Here's how the part is built. I have some questions about the finished solid (model axes, mm). A direction names the side the tool comes from. Give positions to 0.01 mm unless a question says otherwise; leave off trailing zeros. Loops run counter-clockwise (first coordinate to the right, second up) from the corner with the lowest first, then second, coordinate; pieces in that order, holes last.
Q1. I need wall thicknesses on line 1 (Y direction, x = -6.5, z = 0.8); line 2 (Y direction, x = 25, z = 0.2); line 3 (Y direction, x = 34.5, z = 0.2). Which ranges of each line are inside material? Lowest first, please.
Q2. If we section it at D-D (y = 95): Please give me the cut outline in (x, z), plus the area to 3 significant figures.
Q3. For faces 1 (the face through (38.36, 77.6, 0.01)), 2 (the face through (-62.96, 47.39, 0.01)), which set-ups out of +Z, -Z, +X, -X, +Y, -Y let a thin tool reach every point of the face, with its end or its side?
Q4. If we section it at C-C (z = 0.65): Please give me the cut outline in (x, y), plus the area to 3 significant figures.
Q5. We'd pull the mould along Y, two halves only. Please class faces 3 (the face through (-58.7, 104.6, 0)), 4 (the face through (-62.965, 127.462, 0.014)), 5 (the face through (-10, 87, -1)): +Y half, -Y half, draft (parallel to the pull), parting line (faces both ways), or undercut.
Q6. Will this pin go through, and if not, where does the flat tip stop? P1, Ø5, axis at x = -55.5, y = 119.93, coming from the -Z side.
Q7. If we section it at B-B (x = -55.5): Please give me the cut outline in (y, z), plus the area to 3 significant figures.
Q8. If we section it at A-A (x = 24): Please give me the cut outline in (y, z), plus the area to 3 significant figures.
from build123d import *

# Parameters (mm, degrees)
EXTRUDE_1_DEPTH              = 1
HOLE_WIZARD_M6_1_D           = 6.6
HOLE_WIZARD_M6_1_CBORE_D     = 11
HOLE_WIZARD_M6_1_CBORE_DEPTH = 6.4
SKETCH_27_W                  = 153
SKETCH_27_H                  = 120
EXTRUDE_3_DEPTH              = 2
HOLE_WIZARD_M5_2_D           = 4.2
HOLE_WIZARD_M5_2_DEPTH       = 14
HOLE_WIZARD_M5_2_TIP         = 1.2618073
SKETCH_15_W                  = 112.889805259
SKETCH_15_H                  = 130.002769253
CUT_EXTRUDE_1_DEPTH          = 512.721848273
SKETCH_16_R                  = 10
CUT_EXTRUDE_2_DEPTH          = 2
SKETCH_18_R                  = 10
CUT_EXTRUDE_4_DEPTH          = 2
SKETCH_28_W                  = 266.209573984
SKETCH_28_H                  = 254.96875003
CUT_EXTRUDE_7_DEPTH          = 512.721848273
SKETCH_29_W                  = 20
SKETCH_29_H                  = 197
EXTRUDE_4_DEPTH              = 2
SKETCH_30_W                  = 160
SKETCH_30_H                  = 28
EXTRUDE_5_DEPTH              = 2
SKETCH_31_W                  = 160
SKETCH_31_H                  = 323
CUT_EXTRUDE_8_DEPTH          = 471.473431768
SKETCH_32_W                  = 27
SKETCH_32_H                  = 140
CUT_EXTRUDE_9_DEPTH          = 164.022237747
SKETCH_33_R                  = 10
EXTRUDE_6_DEPTH              = 2
EXTRUDE_7_DEPTH              = 2
HOLE_WIZARD_M6_2_D           = 6.6
HOLE_WIZARD_M6_2_CBORE_D     = 11
HOLE_WIZARD_M6_2_CBORE_DEPTH = 6.4
SKETCH_38_W                  = 13
SKETCH_38_H                  = 160
CUT_EXTRUDE_10_DEPTH         = 10
SKETCH_39_W                  = 50
SKETCH_39_H                  = 110.0725
EXTRUDE_8_DEPTH              = 2
SKETCH_40_W                  = 120
SKETCH_40_H                  = 49.9275
CUT_EXTRUDE_11_DEPTH         = 185.727502013
HOLE_WIZARD_5_5_5_5_1_D      = 5.5
MOVE_FACE_1_BY               = 7.5
MOVE_FACE_2_BY               = 7.5
FILLET_4_R                   = 10
SKETCH_44_OUTSIDE_W          = 214.212
SKETCH_44_OUTSIDE_H          = 169.284
SKETCH_44_OUTSIDE_W_2        = 110
SKETCH_44_OUTSIDE_H_2        = 85
CUT_EXTRUDE_12_DEPTH         = 191.47440773
CHAMFER_1_SIZE               = 5
HOLE_WIZARD_5_5_5_5_2_D      = 5.5
CUT_EXTRUDE_13_DEPTH         = 10


with BuildPart() as part:
    # Model → 凸台-拉伸1 (new, symmetric)
    with BuildSketch(Plane.XY):
        with BuildLine():
            Line((186.507023758, 241.511944981), (58.910891188, 92.809685219))
            ThreePointArc((58.910891188, 92.809685219), (57.122071441, 89.769692994), (56.5, 86.297740238))
            Line((56.5, 86.297740238), (56.5, 0))
            Line((56.5, 0), (-73.5, 0))
            ThreePointArc((-73.5, 0), (-80.571067812, 2.928932188), (-83.5, 10))
            Line((-83.5, 10), (-83.5, 335))
            Line((-83.5, 335), (59.5, 335))
            ThreePointArc((59.5, 335), (66.571067812, 337.928932188), (69.5, 345))
            Line((69.5, 345), (69.5, 435))
            Line((69.5, 435), (259.5, 435))
            ThreePointArc((259.5, 435), (266.571067812, 432.071067812), (269.5, 425))
            Line((269.5, 425), (269.5, 255))
            ThreePointArc((269.5, 255), (266.571067812, 247.928932188), (259.5, 245))
            Line((259.5, 245), (194.09613257, 245))
            ThreePointArc((194.09613257, 245), (189.91997703, 244.086238215), (186.507023758, 241.511944981))
        make_face()
    extrude(amount=EXTRUDE_1_DEPTH, both=True)

    # M6 六角凹头螺钉的柱形沉头孔1 (through all)
    with Locations(Plane(origin=(0, 0, -1), x_dir=(-1, 0, 0), z_dir=(0, 0, -1))):
        with Locations((16.5, 157), (-9.5, 235), (-9.5, 157), (16.5, 235)):
            CounterBoreHole(HOLE_WIZARD_M6_1_D / 2, HOLE_WIZARD_M6_1_CBORE_D / 2, HOLE_WIZARD_M6_1_CBORE_DEPTH)

    # 草图27 → 凸台-拉伸3 (add)
    with BuildSketch(Plane.XY.offset(1)):
        with Locations((-7, 375)):
            Rectangle(SKETCH_27_W, SKETCH_27_H)
    extrude(amount=-EXTRUDE_3_DEPTH)

    # M5 螺纹孔2
    with Locations(Plane.XY.offset(1)):
        with Locations((-60.5, 390), (27.5, 405), (47.5, 265), (-32.5, 270)):
            Hole(HOLE_WIZARD_M5_2_D / 2, depth=HOLE_WIZARD_M5_2_DEPTH)
            with Locations((0, 0, -(HOLE_WIZARD_M5_2_DEPTH + HOLE_WIZARD_M5_2_TIP / 2))):  # 118° drill point
                Cone(0, HOLE_WIZARD_M5_2_D / 2, HOLE_WIZARD_M5_2_TIP, mode=Mode.SUBTRACT)

    # 草图15 → 切除-拉伸1 (cut, through all)
    with BuildSketch(Plane.XY.offset(1)):
        with Locations((112.94490263, 131.998615374)):
            Rectangle(SKETCH_15_W, SKETCH_15_H)
    extrude(amount=-CUT_EXTRUDE_1_DEPTH, mode=Mode.SUBTRACT)

    # 草图16 → 切除-拉伸2 (cut)
    with BuildSketch(Plane.XY.offset(1)):
        with Locations((-13.5, 25)):
            Circle(SKETCH_16_R)
    cut_extrude_2 = extrude(amount=-CUT_EXTRUDE_2_DEPTH, mode=Mode.SUBTRACT)

    # 草图18 → 切除-拉伸4 (cut)
    with BuildSketch(Plane.XY.offset(1)):
        with Locations((244.5, 340)):
            Circle(SKETCH_18_R)
    extrude(amount=-CUT_EXTRUDE_4_DEPTH, mode=Mode.SUBTRACT)

    # 草图28 → 切除-拉伸7 (cut, through all)
    with BuildSketch(Plane.XY.offset(1)):
        with Locations((209.604786992, 307.515624985)):
            Rectangle(SKETCH_28_W, SKETCH_28_H)
    extrude(amount=-CUT_EXTRUDE_7_DEPTH, mode=Mode.SUBTRACT)

    # 草图29 → 凸台-拉伸4 (add)
    with BuildSketch(Plane.XY.offset(1)):
        with Locations((66.5, 98.5)):
            Rectangle(SKETCH_29_W, SKETCH_29_H)
    extrude(amount=-EXTRUDE_4_DEPTH)

    # 草图30 → 凸台-拉伸5 (add)
    with BuildSketch(Plane.XY.offset(1)):
        with Locations((-3.5, 449)):
            Rectangle(SKETCH_30_W, SKETCH_30_H)
    extrude(amount=-EXTRUDE_5_DEPTH)

    # 镜向1: 切除-拉伸2 across plane
    add(cut_extrude_2.mirror(Plane.ZX.offset(231.5)), mode=Mode.SUBTRACT)

    # 草图31 → 切除-拉伸8 (cut, through all)
    with BuildSketch(Plane.XY.offset(1)):
        with Locations((-3.5, 301.5)):
            Rectangle(SKETCH_31_W, SKETCH_31_H)
    extrude(amount=-CUT_EXTRUDE_8_DEPTH, mode=Mode.SUBTRACT)

    # 草图32 → 切除-拉伸9 (cut, through all)
    with BuildSketch(Plane.XY.offset(1)):
        with Locations((63, 70)):
            Rectangle(SKETCH_32_W, SKETCH_32_H)
    extrude(amount=-CUT_EXTRUDE_9_DEPTH, mode=Mode.SUBTRACT)

    # 草图33 → 凸台-拉伸6 (add)
    with BuildSketch(Plane.XY.offset(1)):
        with Locations((-13.5, 25)):
            Circle(SKETCH_33_R)
    extrude(amount=-EXTRUDE_6_DEPTH)

    # 草图37 → 凸台-拉伸7 (add)
    with BuildSketch(Plane.XY.offset(1)):
        with BuildLine():
            Line((49.5, 0), (-73.5, 0))
            ThreePointArc((-73.5, 0), (-80.571067812, 2.928932188), (-83.5, 10))
            Line((-83.5, 10), (-83.5, -20))
            Line((-83.5, -20), (49.5, -20))
            Line((49.5, -20), (49.5, 0))
        make_face()
    extrude(amount=-EXTRUDE_7_DEPTH)

    # M6 六角凹头螺钉的柱形沉头孔2 (through all)
    with Locations(Plane.XY.offset(1)):
        with Locations((-40.5, -10), (-40.5, 15), (19.5, 15), (19.5, -10)):
            CounterBoreHole(HOLE_WIZARD_M6_2_D / 2, HOLE_WIZARD_M6_2_CBORE_D / 2, HOLE_WIZARD_M6_2_CBORE_DEPTH)

    # 草图38 → 切除-拉伸10 (cut)
    with BuildSketch(Plane.XY.offset(1)):
        with Locations((-77, 60)):
            Rectangle(SKETCH_38_W, SKETCH_38_H)
    extrude(amount=-CUT_EXTRUDE_10_DEPTH, mode=Mode.SUBTRACT)

    # 草图39 → 凸台-拉伸8 (add)
    with BuildSketch(Plane.XY.offset(1)):
        with Locations((-95.5, 84.96375)):
            Rectangle(SKETCH_39_W, SKETCH_39_H)
    extrude(amount=-EXTRUDE_8_DEPTH)

    # 草图40 → 切除-拉伸11 (cut, through all)
    with BuildSketch(Plane(origin=(0, 0, -1), x_dir=(-1, 0, 0), z_dir=(0, 0, -1))):
        with Locations((10.5, 4.96375)):
            Rectangle(SKETCH_40_W, SKETCH_40_H)
    extrude(amount=-CUT_EXTRUDE_11_DEPTH, mode=Mode.SUBTRACT)

    # Ø5.5 (5.5) 直径孔1 (through all)
    with Locations(Plane.XY.offset(1)):
        with Locations((-87.5, 57.4275), (-112.5, 57.4275), (-112.5, 117.4275), (-87.5, 117.4275)):
            Hole(HOLE_WIZARD_5_5_5_5_1_D / 2)

    # Move Face 1: a face moved outward by 7.5
    extrude(part.faces().sort_by_distance((-35.5, 29.9275, 0))[0], amount=MOVE_FACE_1_BY, dir=(0, -1, 0))

    # Move Face 2: a face moved outward by 7.5
    extrude(part.faces().sort_by_distance((-35.5, 140, 0))[0], amount=MOVE_FACE_2_BY, dir=(0, 1, 0))

    # 圆角4
    fillet_4_edges = [part.edges().sort_by_distance(p)[0] for p in [
        (49.5, 147.5, 0),
        (-120.5, 147.5, 0),
        (-120.5, 22.4275, 0),
        (49.5, 22.4275, 0),
    ]]
    fillet(fillet_4_edges, radius=FILLET_4_R)

    # 草图44 outside → 切除-拉伸12 (cut, through all)
    with BuildSketch(Plane.XY.offset(1)):
        with Locations((-35.5, 84.964)):
            Rectangle(SKETCH_44_OUTSIDE_W, SKETCH_44_OUTSIDE_H)
        with Locations((-10.5, 87.4275)):
            Rectangle(SKETCH_44_OUTSIDE_W_2, SKETCH_44_OUTSIDE_H_2, mode=Mode.SUBTRACT)
    extrude(amount=-CUT_EXTRUDE_12_DEPTH, mode=Mode.SUBTRACT)

    # 倒角1
    chamfer_1_edges = [part.edges().sort_by_distance(p)[0] for p in [
        (-65.5, 129.9275, 0),
        (44.5, 129.9275, 0),
        (44.5, 44.9275, 0),
        (-65.5, 44.9275, 0),
    ]]
    chamfer(chamfer_1_edges, length=CHAMFER_1_SIZE)

    # Ø5.5 (5.5) 直径孔2 (through all)
    with Locations(Plane.XY.offset(1)):
        with Locations((34.5, 54.9275), (34.5, 119.9275), (-55.5, 119.9275), (-55.5, 54.9275)):
            Hole(HOLE_WIZARD_5_5_5_5_2_D / 2)

    # 草图45 → 切除-拉伸13 (cut)
    with BuildSketch(Plane.XY.offset(1)):
        with BuildLine():
            Line((33.36, 72.488602629), (-21.012598119, 72.488602629))
            ThreePointArc((-21.012598119, 72.488602629), (-22.631292343, 72.757870233), (-24.075641802, 73.536671027))
            Line((-24.075641802, 73.536671027), (-57.018167055, 99.06960126))
            ThreePointArc((-57.018167055, 99.06960126), (-58.685855768, 104.640227087), (-53.955123371, 108.021532863))
            Line((-53.955123371, 108.021532863), (0.06, 108.021532863))
            ThreePointArc((0.06, 108.021532863), (5.06, 103.021532863), (0.06, 98.021532863))
            Line((0.06, 98.021532863), (-30.574636438, 98.021532863))
            ThreePointArc((-30.574636438, 98.021532863), (-33.413075876, 95.992749398), (-32.412462648, 92.650373901))
            Line((-32.412462648, 92.650373901), (-19.301769764, 82.488602629))
            Line((-19.301769764, 82.488602629), (33.36, 82.488602629))
            ThreePointArc((33.36, 82.488602629), (38.36, 77.488602629), (33.36, 72.488602629))
        make_face()
    extrude(amount=-CUT_EXTRUDE_13_DEPTH, mode=Mode.SUBTRACT)


solid = part.part
Check sheet entries:
1. line 1: y = 44.93 to 72.49, 82.49 to 98.02, 108.02 to 129.93
1. line 2: y = 44.93 to 72.49, 82.49 to 129.93
1. line 3: y = 44.93 to 52.18, 57.68 to 72.62, 82.36 to 117.18, 122.68 to 129.93
2. outline: (-65.5, -1) - (-51.77, -1) - (-51.77, 1) - (-65.5, 1) - close; (-33.57, -1) - (44.5, -1) - (44.5, 1) - (-33.57, 1) - close
2. area: 184 mm2
3. face 1: +Z, -Z
3. face 2: +Z, -Z, -X, -Y
4. outline: (-65.5, 49.93) - (-60.5, 44.93) - (39.5, 44.93) - (44.5, 49.93) - (44.5, 124.93) - (39.5, 129.93) - (-60.5, 129.93) - (-65.5, 124.93) - close; hole circle Ø5.5 at (-55.5, 54.93); hole circle Ø5.5 at (-55.5, 119.93); hole (-57.02, 99.07) - (-24.08, 73.54) arc R5 ccw to (-21.01, 72.49) - (33.36, 72.49) arc R5 ccw to (33.36, 82.49) - (-19.3, 82.49) - (-32.41, 92.65) arc R3 cw to (-30.57, 98.02) - (0.06, 98.02) arc R5 ccw to (0.06, 108.02) - (-53.96, 108.02) arc R5 ccw to start; hole circle Ø5.5 at (34.5, 54.93); hole circle Ø5.5 at (34.5, 119.93)
4. area: 7,650 mm2
5. face 3: undercut
5. face 4: +Y half
5. face 5: draft
6. P1: passes through
7. outline: (44.93, -1) - (52.18, -1) - (52.18, 1) - (44.93, 1) - close; (57.68, -1) - (97.89, -1) - (97.89, 1) - (57.68, 1) - close; (107.78, -1) - (117.18, -1) - (117.18, 1) - (107.78, 1) - close; (122.68, -1) - (129.93, -1) - (129.93, 1) - (122.68, 1) - close
7. area: 128 mm2
8. outline: (44.93, -1) - (72.49, -1) - (72.49, 1) - (44.93, 1) - close; (82.49, -1) - (129.93, -1) - (129.93, 1) - (82.49, 1) - close
8. area: 150 mm2
